from build123d import *

# Parameters (mm, degrees)
SKETCH1_R           = 15
SKETCH1_R_2         = 9
BOSS_EXTRUDE1_DEPTH = 8
SKETCH2_R           = 13.5
SKETCH2_R_2         = 10.5
CUT_EXTRUDE1_DEPTH  = 6


with BuildPart() as part:
    # Sketch1 → Boss-Extrude1 (new body)
    with BuildSketch(Plane.XY):
        Circle(SKETCH1_R)
        Circle(SKETCH1_R_2, mode=Mode.SUBTRACT)
    extrude(amount=BOSS_EXTRUDE1_DEPTH)

    # Sketch2 → Cut-Extrude1 (cut)
    with BuildSketch(Plane.XY.offset(8)):
        Circle(SKETCH2_R)
        Circle(SKETCH2_R_2, mode=Mode.SUBTRACT)
    extrude(amount=-CUT_EXTRUDE1_DEPTH, mode=Mode.SUBTRACT)


solid = part.part
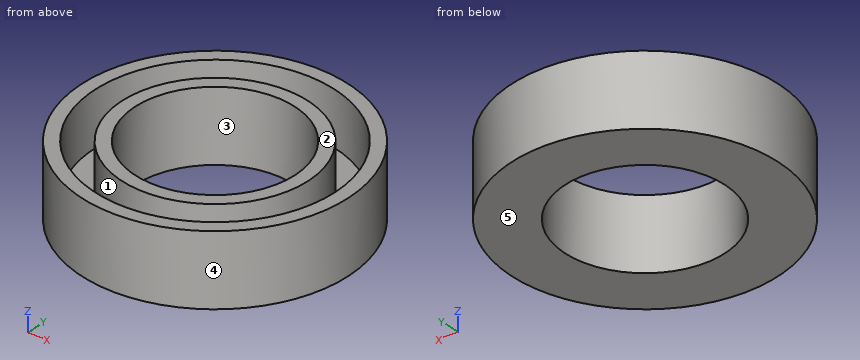
Can you work these out from the model? Positions are in its coordinate system, mm. Face numbers are marked on the shaded views. A direction names the side the tool comes from. Round coordinates to 2 decimals unless told otherwise and drop trailing zeros. Order: outer loops, then holes, each group sorted by start corner. A loop starts at its lowest first (then second) coordinate and runs counter-clockwise, first axis right, second up. Notation, with made-up numbers: (81.25, 85) - (138.25, 85) arc R18 ccw to (138.25, 96) - close; hole circle Ø7 at (-13.5, 12.5). An arc over 180 degrees is marked (long way). Answer in a Markdown table with one row per item.
(1) If we mould it in two halves opening along Y, with no side actions, what happens to the marked faces 3, 4 and 5? For each: released by +Y, released by -Y, zero draft, split by the parting line, or undercut.
From the geometry:
| item | result |
|---|---|
| face 3 | undercut |
| face 4 | split by the parting line |
| face 5 | zero draft |
(2) Suppose I cut it at D-D, the plane z = 1.25. Please give me the cut outline in (x, y), plus the area to 3 significant figures.
From the geometry:
| item | result |
|---|---|
| outline | circle Ø30 at (0, 0); hole circle Ø18 at (0, 0) |
| area | 452 mm2 |
(3) Which directions (+Z, -Z, +X, -X, +Y, -Y) give clear straight access to the entire face, cutting with the end or side of a thin tool? Please do the marked faces 1 and 2.
From the geometry:
| item | result |
|---|---|
| face 1 | +Z |
| face 2 | +Z, +X, -X, +Y, -Y |
(4) Please list where these lines run through material, in increasing order: L1, parallel to Y at x = 0, z = 3.25; L2, parallel to X at y = -0.75, z = 5.25; L3, parallel to X at y = -7.75, z = 5.25. Write a range as from..to.
From the geometry:
| item | result |
|---|---|
| L1 | y = -15..-13.5, -10.5..-9, 9..10.5, 13.5..15 |
| L2 | x = -14.98..-13.48, -10.47..-8.97, 8.97..10.47, 13.48..14.98 |
| L3 | x = -12.84..-11.05, -7.08..-4.58, 4.58..7.08, 11.05..12.84 |
(5) For P1, Ø13.5, axis at x = 3.5, y = -0.5, coming from the +Z side; P2, Ø1, axis at y = -8, z = 5.5, coming from the +X side; P3, Ø1.5, axis at y = 10.5, z = 5.5, coming from the -X side; P4, Ø2, axis at x = -9, z = 5, coming from the -Y side, each with a flat end and sliding along its axis, tell me the tip position at first contact or that it passes through.
From the geometry:
| item | result |
|---|---|
| P1 | stops at z = 8 |
| P2 | stops at x = 12.99 |
| P3 | stops at x = -11.4 |
| P4 | stops at y = -12.69 |
(6) Suppose I cut it at A-A, the plane y = 0. Please give me the cut outline in (x, z), plus the area to 3 significant figures.
From the geometry:
| item | result |
|---|---|
| outline | (-15, 0) - (-9, 0) - (-9, 8) - (-10.5, 8) - (-10.5, 2) - (-13.5, 2) - (-13.5, 8) - (-15, 8) - close; (9, 0) - (15, 0) - (15, 8) - (13.5, 8) - (13.5, 2) - (10.5, 2) - (10.5, 8) - (9, 8) - close |
| area | 60.0 mm2 |
(7) Suppose I cut it at C-C, the plane z = 4. Please give me the cut outline in (x, y), plus the area to 3 significant figures.
From the geometry:
| item | result |
|---|---|
| outline | circle Ø30 at (0, 0); circle Ø21 at (0, 0); hole circle Ø27 at (0, 0); hole circle Ø18 at (0, 0) |
| area | 226 mm2 |
